Geometry: see drawing. Coordinates: mm, zero at the bounding-box minimum. Give positions to 0.01 mm unless a question says otherwise; leave off trailing zeros. Order: outer loops, then holes, each group sorted by start corner. A loop starts at its lowest first (then second) coordinate and runs counter-clockwise, first axis right, second up. Notation, with made-up numbers: (-17.75, 27.5) - (16.25, 27.5) arc R23 cw to (16.25, 52.5) - close; hole circle Ø2 at (4.5, 55.5). An arc over 180 degrees is marked (long way). One line per question, with ' | ' between items. Start each with the question number.
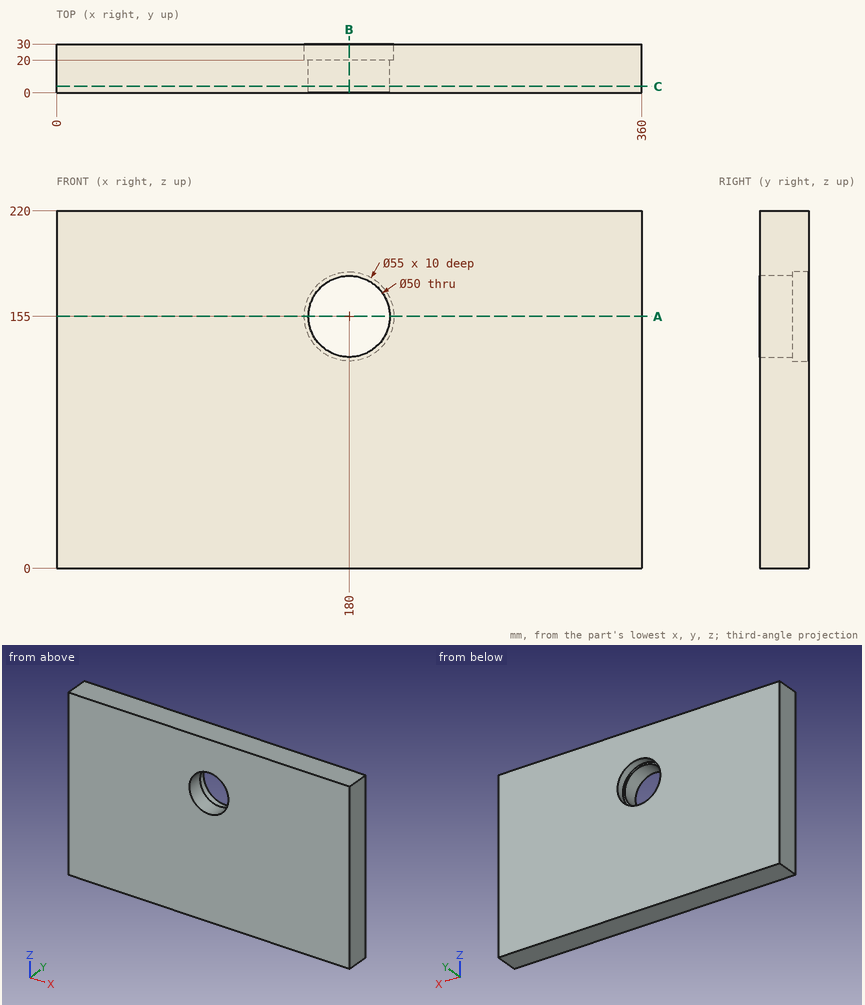
(1) Cut plane C-C, the plane y = 4. Return the cut outline in (x, z), plus the area to 3 significant figures.
(2) Cut plane B-B, the plane x = 180. Return the cut outline in (y, z), plus the area to 3 significant figures.
(3) Cut plane A-A, the plane z = 155. Return the cut outline in (x, y), plus the area to 3 significant figures.
(4) Material intervals for line 1 along X through (y, z) = (4.75, 155); line 2 along Z through (x, y) = (180.5, 9.25) (3 decimals); line 3 along X through (y, z) = (23.5, 155), sorted ascending. Write a range as from..to.
Results are:
1) outline: (0, 0) - (360, 0) - (360, 220) - (0, 220) - close; hole circle Ø50 at (180, 155) | area: 77,200 mm2
2) outline: (0, 0) - (30, 0) - (30, 127.5) - (20, 127.5) - (20, 130) - (0, 130) - close; (0, 180) - (20, 180) - (20, 182.5) - (30, 182.5) - (30, 220) - (0, 220) - close | area: 5,050 mm2
3) outline: (0, 0) - (155, 0) - (155, 20) - (152.5, 20) - (152.5, 30) - (0, 30) - close; (205, 0) - (360, 0) - (360, 30) - (207.5, 30) - (207.5, 20) - (205, 20) - close | area: 9,250 mm2
4) line 1: 0..155, 205..360 | line 2: 0..130.005, 179.995..220 | line 3: 0..152.5, 207.5..360
